Work out the finished part from the listing and answer in its coordinate system (mm). Round coordinates to 2 decimals unless told otherwise and drop trailing zeros. Write each loop counter-clockwise with the first axis right and the second up, starting at its lowest first coordinate (ties: lowest second). Pieces come first, ordered by that corner, then holes.
1. Straight lines are drawn through the part: probe 1 along Y at (x, z) = (0, 4.75); probe 2 along Y at (x, z) = (0, 11.25). For each, find the intervals that lie inside material, in ascending order.
2. Find section A-A (z = 10.25). Write down the section's boundary in (x, y), and give its area (3 significant figures).
3. Flat-ended cylindrical pins translate along their axes: pin 1 Ø6 at (y, z) = (13.5, 6.5) entering from +X; pin 2 Ø1.5 at (x, z) = (34.5, 2) entering from -Y; pin 3 Ø3 at (x, z) = (0.5, 10) entering from -Y. Find the tip coordinate at first contact, or state that the pin passes through.
4. Determine the mould class of faces 1 (the face through (65, -27, 0)), 2 (the face through (-9.764, 74.362, 7.916)), 3 (the face through (50, -50, 2)), 4 (the face through (72.014, 22.678, 7.916)) for opening direction X: pulls with the +X half, pulls with the -X half, needs draft (parallel to the pull), parting line crosses it, or undercut.
5. Find section B-B (y = 0). Write down the section's boundary in (x, z), and give its area (3 significant figures).
```python
from build123d import *

# Parameters (mm, degrees)
SKETCH_1_R               = 75.5
SKETCH_1_R_2             = 75
BOSS_EXTRUDE_1_DEPTH     = 14
SKETCH_2_R               = 75
BOSS_EXTRUDE_2_DEPTH     = 2
CUT_EXTRUDE_1_REACH      = 109.687
SKETCH_3_R               = 70
CUT_EXTRUDE_3_REACH      = 171.403
CUT_EXTRUDE_3_END_RADIUS = 75
CIRCULAR_PATTERN_1_COUNT = 3
FILLET_1_R               = 2


with BuildPart() as part:
    # Sketch 1 → Boss-Extrude 1 (new body)
    with BuildSketch(Plane.XY):
        Circle(SKETCH_1_R)
        Circle(SKETCH_1_R_2, mode=Mode.SUBTRACT)
    extrude(amount=BOSS_EXTRUDE_1_DEPTH)

    # Sketch 2 → Boss-Extrude 2 (add)
    with BuildSketch(Plane.XY):
        Circle(SKETCH_2_R)
    extrude(amount=BOSS_EXTRUDE_2_DEPTH)

    # Sketch 3 → Cut-Extrude 1 (cut, up to next)
    with BuildSketch(Plane(origin=(0, 0, 0), x_dir=(-1, 0, 0), z_dir=(0, 0, -1)), mode=Mode.PRIVATE) as cut_extrude_1_sk1:
        Circle(SKETCH_3_R)
    cut_extrude_1_tool1 = extrude(cut_extrude_1_sk1.sketch, amount=-CUT_EXTRUDE_1_REACH, mode=Mode.PRIVATE) & part.part
    add(cut_extrude_1_tool1.solids().sort_by_distance((0, 0, 0))[0], mode=Mode.SUBTRACT)

    # Cut-Extrude 3: up to this cylinder (the profile starts outside it)
    cut_extrude_3_end = Plane(origin=(0, 0, 9.803668), z_dir=(0, 0, -1)) * Cylinder(CUT_EXTRUDE_3_END_RADIUS, 493.806, mode=Mode.PRIVATE)
    # Sketch 7 → Cut-Extrude 3 (cut, up to the surface)
    with BuildSketch(Plane(origin=(0, 75.5, 0), x_dir=(1, 0, 0), z_dir=(0, 1, 0)), mode=Mode.PRIVATE) as cut_extrude_3_sk1:
        with BuildLine():
            Line((0, -14), (0, -5.25))
            ThreePointArc((0, -5.25), (-1.237436867, -5.762563133), (-1.75, -7))
            Line((-1.75, -7), (-1.75, -14))
            Line((-1.75, -14), (0, -14))
        make_face()
    cut_extrude_3_tool1 = extrude(cut_extrude_3_sk1.sketch, amount=-CUT_EXTRUDE_3_REACH, mode=Mode.PRIVATE) - cut_extrude_3_end
    # Sketch 7 → Cut-Extrude 3 (cut, up to the surface)
    with BuildSketch(Plane(origin=(0, 75.5, 0), x_dir=(1, 0, 0), z_dir=(0, 1, 0)), mode=Mode.PRIVATE) as cut_extrude_3_sk2:
        with BuildLine():
            ThreePointArc((1.75, -7), (1.237436867, -5.762563133), (0, -5.25))
            Line((0, -5.25), (0, -14))
            Line((0, -14), (1.75, -14))
            Line((1.75, -14), (1.75, -7))
        make_face()
    cut_extrude_3_tool2 = extrude(cut_extrude_3_sk2.sketch, amount=-CUT_EXTRUDE_3_REACH, mode=Mode.PRIVATE) - cut_extrude_3_end
    cut_extrude_3 = cut_extrude_3_tool1.solids().sort_by_distance((-0.85329, 75.5, 9.803668))[0] + cut_extrude_3_tool2.solids().sort_by_distance((0.85329, 75.5, 9.803668))[0]
    add(cut_extrude_3, mode=Mode.SUBTRACT)

    # Circular pattern 1: Cut-Extrude 3 ×3 about axis
    circular_pattern_1_axis = Axis((0, 0, 0), (0, 0, 1))
    for i in range(1, CIRCULAR_PATTERN_1_COUNT):
        add(cut_extrude_3.rotate(circular_pattern_1_axis, i * 360 / CIRCULAR_PATTERN_1_COUNT), mode=Mode.SUBTRACT)

    # Fillet 1
    fillet_1_edges = [part.edges().sort_by_distance(p)[0] for p in [
        (-75.5, 0, 0),
    ]]
    fillet(fillet_1_edges, radius=FILLET_1_R)


solid = part.part
```
Worked answers:
1. probe 1: y = -75.5 to -75, 75 to 75.5
1. probe 2: y = -75.5 to -75
2. outline: (-66.24, -36.22) - (-65.81, -35.97) arc R75 cw to (-1.75, 74.98) - (-1.75, 75.48) arc R75.5 ccw to start; (-64.49, -39.26) arc R75.5 ccw to (64.49, -39.26) - (64.06, -39.01) arc R75 cw to (-64.06, -39.01) - close; (1.75, 74.98) arc R75 cw to (65.81, -35.97) - (66.24, -36.22) arc R75.5 ccw to (1.75, 75.48) - close
2. area: 231 mm2
3. pin 1: stops at x = 74.77
3. pin 2: stops at y = -67.54
3. pin 3: stops at y = -75.5
4. face 1: needs draft
4. face 2: undercut
4. face 3: undercut
4. face 4: parting line crosses it
5. outline: (-75.5, 2) arc R2 ccw to (-73.5, 0) - (-70, 0) - (-70, 2) - (-75, 2) - (-75, 14) - (-75.5, 14) - close; (70, 0) - (73.5, 0) arc R2 ccw to (75.5, 2) - (75.5, 14) - (75, 14) - (75, 2) - (70, 2) - close
5. area: 32.3 mm2
